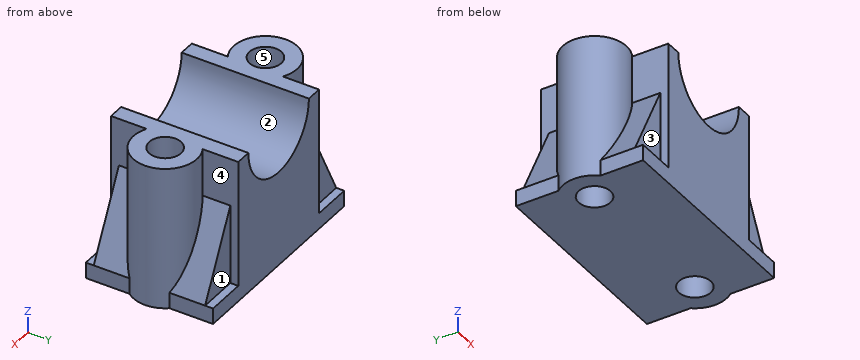
```python
from build123d import *

# Parameters (mm, degrees)
BASE_PLATE_SKETCH_W    = 130
BASE_PLATE_SKETCH_H    = 80
BASE_PLATE_10MM_DEPTH  = 10
MAIN_BODY_PROFILE_W    = 10
MAIN_BODY_PROFILE_H    = 80
MAIN_BODY_DEPTH        = 80
SIDE_WALL_A_DEPTH      = 90
SIDE_WALL_B_DEPTH      = 90
HALF_BORE_SKETCH_R     = 10
HALF_BORE_CUT_DEPTH    = 90
RIB_A_DEPTH            = 28
RIB_B_DEPTH            = 28
BOSS_DEPTH             = 28
RECESS_CUT_A_5MM_DEPTH = 5
RECESS_CUT_B_5MM_DEPTH = 5


with BuildPart() as part:
    # Base Plate Sketch → Base Plate 10mm (new body)
    with BuildSketch(Plane.XY):
        with Locations((65, 40)):
            Rectangle(BASE_PLATE_SKETCH_W, BASE_PLATE_SKETCH_H)
    extrude(amount=BASE_PLATE_10MM_DEPTH)

    # Main Body Profile → Main Body (add)
    with BuildSketch(Plane.XZ):
        with Locations((30, 50)):
            Rectangle(MAIN_BODY_PROFILE_W, MAIN_BODY_PROFILE_H)
        with BuildLine():
            Line((35, 10), (65, 10))
            Line((65, 10), (95, 10))
            Line((95, 10), (95, 90))
            ThreePointArc((95, 90), (65, 60), (35, 90))
            Line((35, 90), (35, 10))
        make_face()
        with Locations((100, 50)):
            Rectangle(MAIN_BODY_PROFILE_W, MAIN_BODY_PROFILE_H)
    extrude(amount=-MAIN_BODY_DEPTH)

    # Side Wall A Sketch → Side Wall A (add)
    with BuildSketch(Plane.XY.offset(90)):
        with BuildLine():
            Line((105, 57.643408065), (105, 22.356591935))
            ThreePointArc((105, 22.356591935), (134.418606683, 40), (105, 57.643408065))
        make_face()
    extrude(amount=-SIDE_WALL_A_DEPTH)

    # Side Wall B Sketch → Side Wall B (add)
    with BuildSketch(Plane.XY.offset(90)):
        with BuildLine():
            Line((25, 57.320508076), (25, 22.679491924))
            ThreePointArc((25, 22.679491924), (-5, 40), (25, 57.320508076))
        make_face()
    extrude(amount=-SIDE_WALL_B_DEPTH)

    # Half Bore Sketch → Half Bore Cut (cut)
    with BuildSketch(Plane.XY.offset(90)):
        with Locations((114.418606683, 40)):
            Circle(HALF_BORE_SKETCH_R)
        with Locations((15, 40)):
            Circle(HALF_BORE_SKETCH_R)
    extrude(amount=-HALF_BORE_CUT_DEPTH, mode=Mode.SUBTRACT)

    # Rib A Sketch → Rib A (add)
    with BuildSketch(Plane.XZ):
        Polygon((105, 10), (105, 60), (130, 10), align=None)
    extrude(amount=-RIB_A_DEPTH)

    # Rib B Sketch → Rib B (add)
    with BuildSketch(Plane.XZ):
        Polygon((25, 10), (25, 60), (0, 10), align=None)
    extrude(amount=-RIB_B_DEPTH)

    # Boss Sketch → Boss (add)
    with BuildSketch(Plane(origin=(0, 80, 0), x_dir=(1, 0, 0), z_dir=(0, 1, 0))):
        Polygon((105, -10), (105, -60), (130, -10), align=None)
        Polygon((25, -10), (25, -60), (0, -10), align=None)
    extrude(amount=-BOSS_DEPTH)

    # Recess A Sketch → Recess Cut A 5mm (cut)
    with BuildSketch(Plane.XZ):
        Polygon((25, 60), (25, 10), (0, 10), align=None)
        Polygon((105, 60), (105, 10), (130, 10), align=None)
    extrude(amount=-RECESS_CUT_A_5MM_DEPTH, mode=Mode.SUBTRACT)

    # Recess B Sketch → Recess Cut B 5mm (cut)
    with BuildSketch(Plane(origin=(0, 80, 0), x_dir=(1, 0, 0), z_dir=(0, 1, 0))):
        Polygon((25, -60), (25, -10), (0, -10), align=None)
        Polygon((105, -60), (105, -10), (130, -10), align=None)
    extrude(amount=-RECESS_CUT_B_5MM_DEPTH, mode=Mode.SUBTRACT)


solid = part.part
```
CAD build for the part. Positions are in the model's coordinates, mm. Face numbers are marked on the shaded views. A direction names the side the tool comes from. Coordinates: 2 decimals unless noted, no trailing zeros. Write each loop counter-clockwise with the first axis right and the second up, starting at its lowest first coordinate (ties: lowest second). Pieces come first, ordered by that corner, then holes. Notation, with made-up numbers: (78, 58.25) -> (84, 58.25) arc R5 ccw to (84, 62.25) -> close; hole circle Ø7 at (49, 2.5). An arc over 180 degrees is marked (long way). Use CSV: the item, a comma, the result in double quotes. Start each with the question number.
Item 1: Band-saw the part on C-C, the plane y = 40. Write the cut outline in (x, z), plus the area to 3 significant figures.
Item 2: Drop flat-ended pins along their axis: P1, Ø7, axis at y = 69.5, z = 60, coming from the -X side; P2, Ø2, axis at x = 14.5, z = 80, coming from the -Y side; P3, Ø6, axis at x = 62.5, y = 29.5, coming from the +Z side. Give the stop position or say it passes through.
Item 3: Two-plate mould, pull along Y, no slides. Class the marked faces 3, 4 and 5: +Y half, -Y half, draft (parallel to the pull), parting line (faces both ways), or undercut.
Item 4: Tool access for the marked faces 1 and 2: list every direction of +Z, -Z, +X, -X, +Y, -Y with a clear straight run to the whole face (end or side of a thin tool).
Item 5: Wall check: probe 1 along Y at (x, z) = (15, 52); probe 2 along X at (y, z) = (47.5, 42.5); probe 3 along Z at (x, y) = (65, 23). Give the ranges that are in metal, low to high.
Item 6: Band-saw the part on D-D, the plane z = 20. Write the cut outline in (x, y), plus the area to 3 significant figures.
Item 7: Band-saw the part on A-A, the plane x = 15. Write the cut outline in (y, z), plus the area to 3 significant figures.
Item 8: Band-saw the part on B-B, the plane z = 61.5. Write the cut outline in (x, y), plus the area to 3 significant figures.
Response values:
1,outline,"(-5, 0) -> (5, 0) -> (5, 90) -> (-5, 90) -> close; (25, 0) -> (104.42, 0) -> (104.42, 90) -> (95, 90) arc R30 cw to (35, 90) -> (25, 90) -> close; (124.42, 0) -> (134.42, 0) -> (134.42, 90) -> (124.42, 90) -> close"
1,area,"7,530 mm2"
2,P1,"stops at x = 23.25"
2,P2,"stops at y = 20"
2,P3,"stops at z = 60.51"
3,face 3,"-Y half"
3,face 4,"draft"
3,face 5,"undercut"
4,face 1,"+Z, +X, +Y"
4,face 2,"+Z, +Y, -Y"
5,probe 1,"y = 20 to 30, 50 to 60"
5,probe 2,"x = -3.54 to 8.39, 21.61 to 107.8, 121.03 to 132.96"
5,probe 3,"z = 0 to 60"
6,outline,"(5, 5) -> (25, 5) -> (25, 0) -> (105, 0) -> (105, 5) -> (125, 5) -> (125, 23.03) arc R20 ccw to (125, 56.97) -> (125, 75) -> (105, 75) -> (105, 80) -> (25, 80) -> (25, 75) -> (5, 75) -> (5, 57.32) arc R20 ccw to (5, 22.68) -> close; hole circle Ø20 at (15, 40); hole circle Ø20 at (114.42, 40)"
6,area,"9,040 mm2"
7,outline,"(0, 0) -> (30, 0) -> (30, 90) -> (20, 90) -> (20, 40) -> (5, 40) -> (5, 10) -> (0, 10) -> close; (50, 0) -> (80, 0) -> (80, 10) -> (75, 10) -> (75, 40) -> (60, 40) -> (60, 90) -> (50, 90) -> close"
7,area,"3,100 mm2"
8,outline,"(25, 0) -> (55.63, 0) -> (55.63, 80) -> (25, 80) -> (25, 57.32) arc R20 ccw (long way) to (25, 22.68) -> close; (74.37, 0) -> (105, 0) -> (105, 22.36) arc R20 ccw (long way) to (105, 57.64) -> (105, 80) -> (74.37, 80) -> close; hole circle Ø20 at (15, 40); hole circle Ø20 at (114.42, 40)"
8,area,"6,270 mm2"
